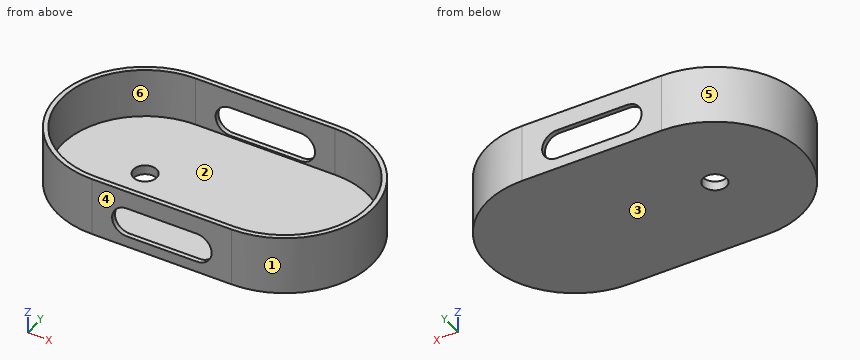
```python
from build123d import *

# Parameters (mm, degrees)
SKETCH1_R           = 5
BOSS_EXTRUDE1_DEPTH = 25
CUT_EXTRUDE1_DEPTH  = 21
CUT_EXTRUDE2_DEPTH  = 21


with BuildPart() as part:
    # Sketch1 → Boss-Extrude1 (new body)
    with BuildSketch(Plane.XY):
        with BuildLine():
            Line((0, 37.5), (60, 37.5))
            ThreePointArc((60, 37.5), (97.5, 0), (60, -37.5))
            Line((60, -37.5), (0, -37.5))
            ThreePointArc((0, -37.5), (-37.5, 0), (0, 37.5))
        make_face()
        Circle(SKETCH1_R, mode=Mode.SUBTRACT)
    extrude(amount=BOSS_EXTRUDE1_DEPTH)

    # Sketch2 → Cut-Extrude1 (cut)
    with BuildSketch(Plane.XY.offset(25)):
        with BuildLine():
            Line((60, 35.5), (0, 35.5))
            ThreePointArc((0, 35.5), (-35.5, 0), (0, -35.5))
            Line((0, -35.5), (60, -35.5))
            ThreePointArc((60, -35.5), (95.5, 0), (60, 35.5))
        make_face()
    extrude(amount=-CUT_EXTRUDE1_DEPTH, mode=Mode.SUBTRACT)

    # Sketch4 → Cut-Extrude2 (cut)
    with BuildSketch(Plane.XZ.offset(37.5)):
        with BuildLine():
            Line((15, 17.341846587), (45, 17.341846587))
            ThreePointArc((45, 17.341846587), (51.341846587, 11), (45, 4.658153413))
            Line((45, 4.658153413), (15, 4.658153413))
            ThreePointArc((15, 4.658153413), (8.658153413, 11), (15, 17.341846587))
        make_face()
    cut_extrude2 = extrude(amount=-CUT_EXTRUDE2_DEPTH, mode=Mode.SUBTRACT)

    # Mirror2: Cut-Extrude2 across plane
    add(cut_extrude2.mirror(Plane.ZX), mode=Mode.SUBTRACT)


solid = part.part
```
Can you work these out from the model? Positions are in its coordinate system, mm. Face numbers are marked on the shaded views. A direction names the side the tool comes from. Round coordinates to 2 decimals unless told otherwise and drop trailing zeros. Loops run counter-clockwise (first coordinate to the right, second up) from the corner with the lowest first, then second, coordinate; pieces in that order, holes last.
Item 1: Suppose I cut it at B-B, the plane y = 0. Write out the boundary of the cut face in (x, z).
Item 2: Suppose I cut it at D-D, the plane x = 3. Write out the boundary of the cut face in (y, z).
Item 3: Will these pins go through, and if not, where does the flat tip stop? pin 1 Ø1 at (y, z) = (25, 11) entering from +X; pin 2 Ø1 at (y, z) = (-7, 11) entering from +X; pin 3 Ø10 at (y, z) = (10.5, 21) entering from +X.
Item 4: If we mould it in two halves opening along Y, with no side actions, what happens to the marked faces 1, 2, 3 and 4? For each: +Y half, -Y half, draft (parallel to the pull), parting line (faces both ways), or undercut.
Item 5: Which directions (+Z, -Z, +X, -X, +Y, -Y) give clear straight access to the entire face, cutting with the end or side of a thin tool? Please do the marked faces 5 and 6.
Item 6: Suppose I cut it at C-C, the plane x = 40. Write out the boundary of the cut face in (y, z), then the cut area to 3 significant figures.
Item 7: Suppose I cut it at A-A, the plane z = 11. Write out the boundary of the cut face in (x, y), then the cut area to 3 significant figures.
Item 8: Please list where these lines run through material, in increasing order: L1, parallel to Y at x = 0, z = 2.7; L2, parallel to Y at x = 37.5, z = 4.5; L3, parallel to X at y = 0, z = 2.5.
Reported:
1. outline: (-37.5, 0) - (-5, 0) - (-5, 4) - (-35.5, 4) - (-35.5, 25) - (-37.5, 25) - close; (5, 0) - (97.5, 0) - (97.5, 25) - (95.5, 25) - (95.5, 4) - (5, 4) - close
2. outline: (-37.5, 0) - (-4, 0) - (-4, 4) - (-35.5, 4) - (-35.5, 25) - (-37.5, 25) - close; (4, 0) - (37.5, 0) - (37.5, 25) - (35.5, 25) - (35.5, 4) - (4, 4) - close
3. pin 1: stops at x = 88.39
3. pin 2: stops at x = 96.93
3. pin 3: stops at x = 97.09
4. face 1: parting line
4. face 2: undercut
4. face 3: draft
4. face 4: -Y half
5. face 5: +Z, -Z, -X
5. face 6: +Z
6. outline: (-37.5, 0) - (37.5, 0) - (37.5, 4.66) - (35.5, 4.66) - (35.5, 4) - (-35.5, 4) - (-35.5, 4.66) - (-37.5, 4.66) - close; (-37.5, 17.34) - (-35.5, 17.34) - (-35.5, 25) - (-37.5, 25) - close; (35.5, 17.34) - (37.5, 17.34) - (37.5, 25) - (35.5, 25) - close
6. area: 333 mm2
7. outline: (0, -37.5) - (8.66, -37.5) - (8.66, -35.5) - (0, -35.5) arc R35.5 cw to (0, 35.5) - (8.66, 35.5) - (8.66, 37.5) - (0, 37.5) arc R37.5 ccw to start; (51.34, -37.5) - (60, -37.5) arc R37.5 ccw to (60, 37.5) - (51.34, 37.5) - (51.34, 35.5) - (60, 35.5) arc R35.5 cw to (60, -35.5) - (51.34, -35.5) - close
7. area: 528 mm2
8. L1: y = -37.5 to -5, 5 to 37.5
8. L2: y = -37.5 to -35.5, 35.5 to 37.5
8. L3: x = -37.5 to -5, 5 to 97.5
